```python
from build123d import *

# Parameters (mm, degrees)
BOSS_EXTRUDE1_DEPTH = 10
FILLET1_R           = 20
CHAMFER1_SIZE       = 20


with BuildPart() as part:
    # Sketch1 → Boss-Extrude1 (new, symmetric)
    with BuildSketch(Plane.XY):
        Polygon((0, 0), (314, 0), (314, 140), (50, 600), (0, 600), align=None)
    extrude(amount=BOSS_EXTRUDE1_DEPTH, both=True)

    # Fillet1
    fillet1_edges = [part.edges().sort_by_distance(p)[0] for p in [
        (50, 600, 0),
    ]]
    fillet(fillet1_edges, radius=FILLET1_R)

    # Chamfer1
    chamfer1_edges = [part.edges().sort_by_distance(p)[0] for p in [
        (314, 0, 0),
        (0, 0, 0),
    ]]
    chamfer(chamfer1_edges, length=CHAMFER1_SIZE)


solid = part.part
```
The listing builds one solid part. Answer for the finished solid, in the listing's coordinates (mm). Round coordinates to 2 decimals unless told otherwise and drop trailing zeros. Order: outer loops, then holes, each group sorted by start corner. A loop starts at its lowest first (then second) coordinate and runs counter-clockwise, first axis right, second up. Notation, with made-up numbers: (69, 58) -> (125, 58) arc R19 cw to (125, 95) -> close; hole circle Ø11 at (-37.75, -37). An arc over 180 degrees is marked (long way). Answer as CSV lines item,"result".
Q1. A cutting plane is placed at A-A on z = -1.5. Determine the outline of the cut face in (x, y), plus the area to 3 significant figures.
Computed values:
outline,"(0, 20) -> (20, 0) -> (294, 0) -> (314, 20) -> (314, 140) -> (55.76, 589.96) arc R20 ccw to (38.42, 600) -> (0, 600) -> close"
area,"127,000 mm^2"
Q2. Given pin 1 (5 mm diameter, centred on y = 205, z = 2, fed in from +X); pin 2 (2 mm diameter, centred on x = 263.5, z = 4.5, fed in from +Y); pin 3 (3 mm diameter, centred on y = 396, z = -5, fed in from +X), each flat-ended and moving along its own axis, determine where each tip first touches the part or whether it passes through.
Computed values:
pin 1,"stops at x = 278.13"
pin 2,"stops at y = 229.73"
pin 3,"stops at x = 167.94"
Q3. Consider line 1 (X direction, y = 456.5, z = -9); line 2 (Y direction, x = 91.5, z = 5.75); line 3 (Y direction, x = 162.5, z = -5.75). Determine where each line is inside the solid, lowest interval first. Write a range as from..to.
Computed values:
line 1,"x = 0..132.36"
line 2,"y = 0..527.69"
line 3,"y = 0..403.98"
Q4. A cutting plane is placed at C-C on x = 245.5. Determine the outline of the cut face in (y, z), plus the area to 3 significant figures.
Computed values:
outline,"(0, -10) -> (259.36, -10) -> (259.36, 10) -> (0, 10) -> close"
area,"5,190 mm^2"
Q5. A cutting plane is placed at B-B on y = 467. Determine the outline of the cut face in (x, z).
Computed values:
outline,"(0, -10) -> (126.33, -10) -> (126.33, 10) -> (0, 10) -> close"
